from build123d import *

# Parameters (mm, degrees)
SKETCH1_R           = 11.15
SKETCH1_R_2         = 1.7
SKETCH1_R_3         = 1
SKETCH1_R_4         = 2.5
BOSS_EXTRUDE1_DEPTH = 8
SKETCH2_R           = 4.5
CUT_EXTRUDE1_DEPTH  = 5.5
SKETCH3_R           = 3
CUT_EXTRUDE2_DEPTH  = 4
CHAMFER1_SIZE       = 1
CHAMFER2_SIZE       = 0.5
CHAMFER3_SIZE       = 0.5
SKETCH4_R           = 19
CUT_EXTRUDE3_DEPTH  = 2
CUT_EXTRUDE4_DEPTH  = 1
CHAMFER4_SIZE       = 1
M4_TAPPED_HOLE1_D   = 3.3
CHAMFER5_SIZE       = 0.5


with BuildPart() as part:
    # Sketch1 → Boss-Extrude1 (new body)
    with BuildSketch(Plane.XY):
        with BuildLine():
            Line((-27, 35.5), (27, 35.5))
            ThreePointArc((27, 35.5), (27.707106781, 35.207106781), (28, 34.5))
            Line((28, 34.5), (28, -35.5))
            Line((28, -35.5), (-28, -35.5))
            Line((-28, -35.5), (-28, 34.5))
            ThreePointArc((-28, 34.5), (-27.707106781, 35.207106781), (-27, 35.5))
        make_face()
        with Locations((0, 7)):
            Circle(SKETCH1_R, mode=Mode.SUBTRACT)
        with Locations((-15.55, 22.55)):
            Circle(SKETCH1_R_2, mode=Mode.SUBTRACT)
        with Locations((-23.55, 30.55)):
            Circle(SKETCH1_R_3, mode=Mode.SUBTRACT)
        with Locations(Location((23.55, 30.55, 0), (0, 0, 180))):
            Circle(SKETCH1_R_3, mode=Mode.SUBTRACT)
        with Locations(Location((15.55, 22.55, 0), (0, 0, 180))):
            Circle(SKETCH1_R_2, mode=Mode.SUBTRACT)
        with Locations(Location((-23.55, -16.55, 0), (0, 0, 180))):
            Circle(SKETCH1_R_3, mode=Mode.SUBTRACT)
        with Locations(Location((-15.55, -8.55, 0), (0, 0, 180))):
            Circle(SKETCH1_R_2, mode=Mode.SUBTRACT)
        with Locations((15.55, -8.55)):
            Circle(SKETCH1_R_2, mode=Mode.SUBTRACT)
        with Locations((23.55, -16.55)):
            Circle(SKETCH1_R_3, mode=Mode.SUBTRACT)
        with Locations((-15, -25.5)):
            Circle(SKETCH1_R_4, mode=Mode.SUBTRACT)
        with Locations((15, -25.5)):
            Circle(SKETCH1_R_4, mode=Mode.SUBTRACT)
    extrude(amount=BOSS_EXTRUDE1_DEPTH)

    # Sketch2 → Cut-Extrude1 (cut)
    with BuildSketch(Plane.XY.offset(8)):
        with Locations((-15, -25.5)):
            Circle(SKETCH2_R)
        with Locations((15, -25.5)):
            Circle(SKETCH2_R)
    extrude(amount=-CUT_EXTRUDE1_DEPTH, mode=Mode.SUBTRACT)

    # Sketch3 → Cut-Extrude2 (cut)
    with BuildSketch(Plane(origin=(0, 0, 0), x_dir=(-1, 0, 0), z_dir=(0, 0, -1))):
        with Locations((-15.55, 22.55)):
            Circle(SKETCH3_R)
        with Locations((15.55, 22.55)):
            Circle(SKETCH3_R)
        with Locations((-15.55, -8.55)):
            Circle(SKETCH3_R)
        with Locations((15.55, -8.55)):
            Circle(SKETCH3_R)
    extrude(amount=-CUT_EXTRUDE2_DEPTH, mode=Mode.SUBTRACT)

    # Chamfer1
    chamfer1_edges = [part.edges().sort_by_distance(p)[0] for p in [
        (18.55, 22.55, 0),
        (-12.55, 22.55, 0),
        (18.55, -8.55, 0),
        (-12.55, -8.55, 0),
    ]]
    chamfer(chamfer1_edges, length=CHAMFER1_SIZE)

    # Chamfer2
    chamfer2_edges = [part.edges().sort_by_distance(p)[0] for p in [
        (-24.55, 30.55, 0),
        (24.55, 30.55, 0),
        (-22.55, -16.55, 0),
        (22.55, -16.55, 0),
    ]]
    chamfer(chamfer2_edges, length=CHAMFER2_SIZE)

    # Chamfer3
    chamfer3_edges = [part.edges().sort_by_distance(p)[0] for p in [
        (-24.55, 30.55, 8),
        (24.55, 30.55, 8),
        (-22.55, -16.55, 8),
        (22.55, -16.55, 8),
    ]]
    chamfer(chamfer3_edges, length=CHAMFER3_SIZE)

    # Sketch4 → Cut-Extrude3 (cut)
    with BuildSketch(Plane.XY.offset(8)):
        with Locations((0, 7)):
            Circle(SKETCH4_R)
    extrude(amount=-CUT_EXTRUDE3_DEPTH, mode=Mode.SUBTRACT)

    # Sketch5 → Cut-Extrude4 (cut)
    with BuildSketch(Plane.XY.offset(8)):
        with BuildLine():
            Line((-13.5, 28.5), (13.5, 28.5))
            ThreePointArc((13.5, 28.5), (19.156854249, 26.156854249), (21.5, 20.5))
            Line((21.5, 20.5), (21.5, -6.5))
            ThreePointArc((21.5, -6.5), (19.156854249, -12.156854249), (13.5, -14.5))
            Line((13.5, -14.5), (-13.5, -14.5))
            ThreePointArc((-13.5, -14.5), (-19.156854249, -12.156854249), (-21.5, -6.5))
            Line((-21.5, -6.5), (-21.5, 20.5))
            ThreePointArc((-21.5, 20.5), (-19.156854249, 26.156854249), (-13.5, 28.5))
        make_face()
    extrude(amount=-CUT_EXTRUDE4_DEPTH, mode=Mode.SUBTRACT)

    # Chamfer4
    chamfer4_edges = [part.edges().sort_by_distance(p)[0] for p in [
        (-19.5, -25.5, 8),
        (10.5, -25.5, 8),
    ]]
    chamfer(chamfer4_edges, length=CHAMFER4_SIZE)

    # M4 Tapped Hole1 (through all)
    with Locations(Plane.XY.offset(8)):
        with Locations((-23.55, 30.55), (23.55, 30.55), (23.55, -16.55), (-23.55, -16.55)):
            Hole(M4_TAPPED_HOLE1_D / 2)

    # Chamfer5
    chamfer5_edges = [part.edges().sort_by_distance(p)[0] for p in [
        (-21.9, -16.55, 8),
        (-21.9, -16.55, 0),
        (25.2, -16.55, 8),
        (25.2, -16.55, 0),
        (25.2, 30.55, 8),
        (25.2, 30.55, 0),
        (-21.9, 30.55, 8),
        (-21.9, 30.55, 0),
    ]]
    chamfer(chamfer5_edges, length=CHAMFER5_SIZE)


solid = part.part
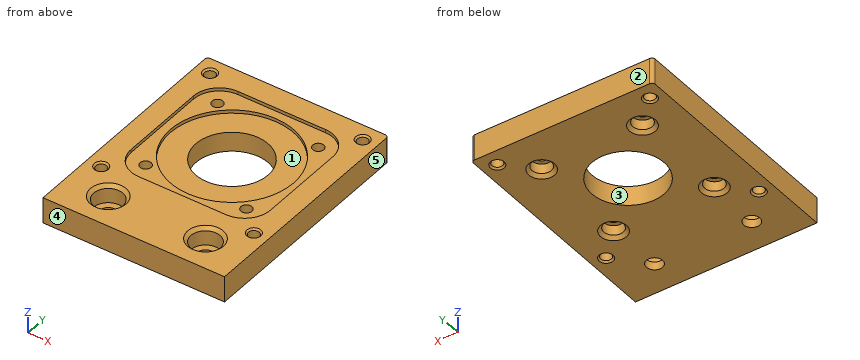
Input: part model. Units: mm. Frame: model coordinates. Face numbers are marked on the shaded views. A direction names the side the tool comes from. Coordinates: 2 decimals unless noted, no trailing zeros. Order: outer loops, then holes, each group sorted by start corner. A loop starts at its lowest first (then second) coordinate and runs counter-clockwise, first axis right, second up. Notation, with made-up numbers: M 24.5,84 L 73.5,84 A14 cw 73.5,104 Z; hole C -19.5,-29.75 d4. An arc over 180 degrees is marked long. Write item = value, one per line. Start each with the question number.
(1) Line query: line 1 along X through (y, z) = (-16.5, 5); line 2 along X through (y, z) = (-8, 1.75); line 3 along Y through (x, z) = (17, 4.5). Output: solid intervals per line, ascending. Write a range as [from, to].
(2) Section B-B on y = -25.5. Output: boundary loops of the cut face in (x, z).
(3) Pull-direction query (Y, two-part tool) for the marked faces 3, 4 and 5; classes: released by +Y, released by -Y, zero draft, split by the parting line, or undercut.
(4) First-contact query: P1, Ø5.5, axis at x = 15.55, y = -8.55, coming from the +Z side; P2, Ø7, axis at x = 14.5, y = -25, coming from the +Z side; P3, Ø4.5, axis at x = -13.5, y = -23.5, coming from the +Z side. Flat tips, straight axial feed; report the tip coordinate or a pass-through.
(5) Section D-D on x = -16. Give the number of separate pieces and of enclosed holes in the cut face, and give its area (3 significant figures).
(6) Section C-C on y = 30.55. Output: boundary loops of the cut face in (x, z), and give its area (3 significant figures).
(7) Section A-A on y = 7. Output: boundary loops of the cut face in (x, z), and give its area (3 significant figures).
(8) Reachability of the marked faces 1 and 2 from +Z, -Z, +X, -X, +Y, -Y: full face, straight path, thin tool, end or side. Return the list, or none.
Result set:
q1.line_1 = [-28, -25.2], [-21.9, 21.9], [25.2, 28]
q1.line_2 = [-28, -18.5], [-12.6, 12.6], [18.5, 28]
q1.line_3 = [-35.5, -29.53], [-21.47, -9.44], [-7.66, 21.66], [23.44, 35.5]
q2.outline = M -28,0 L -17.5,0 L -17.5,2.5 L -19.5,2.5 L -19.5,7 L -20.5,8 L -28,8 Z; M -12.5,0 L 12.5,0 L 12.5,2.5 L 10.5,2.5 L 10.5,7 L 9.5,8 L -9.5,8 L -10.5,7 L -10.5,2.5 L -12.5,2.5 Z; M 17.5,0 L 28,0 L 28,8 L 20.5,8 L 19.5,7 L 19.5,2.5 L 17.5,2.5 Z
q3.face_3 = undercut
q3.face_4 = released by -Y
q3.face_5 = zero draft
q4.P1 = 7
q4.P2 = 2.5
q4.P3 = 7.25
q5.separate_pieces = 4
q5.enclosed_holes = 0
q5.area = 375 mm²
q6.outline = M -28,0 L -25.7,0 L -25.2,0.5 L -25.2,7.5 L -25.7,8 L -28,8 Z; M -21.9,0.5 L -21.4,0 L 21.4,0 L 21.9,0.5 L 21.9,7.5 L 21.4,8 L -21.4,8 L -21.9,7.5 Z; M 25.2,0.5 L 25.7,0 L 28,0 L 28,8 L 25.7,8 L 25.2,7.5 Z
q6.area = 394 mm²
q7.outline = M -28,0 L -11.15,0 L -11.15,6 L -19,6 L -19,7 L -21.5,7 L -21.5,8 L -28,8 Z; M 11.15,0 L 28,0 L 28,8 L 21.5,8 L 21.5,7 L 19,7 L 19,6 L 11.15,6 Z
q7.area = 233 mm²
q8.face_1 = +Z
q8.face_2 = +Z, -Z, +X, -X, +Y
